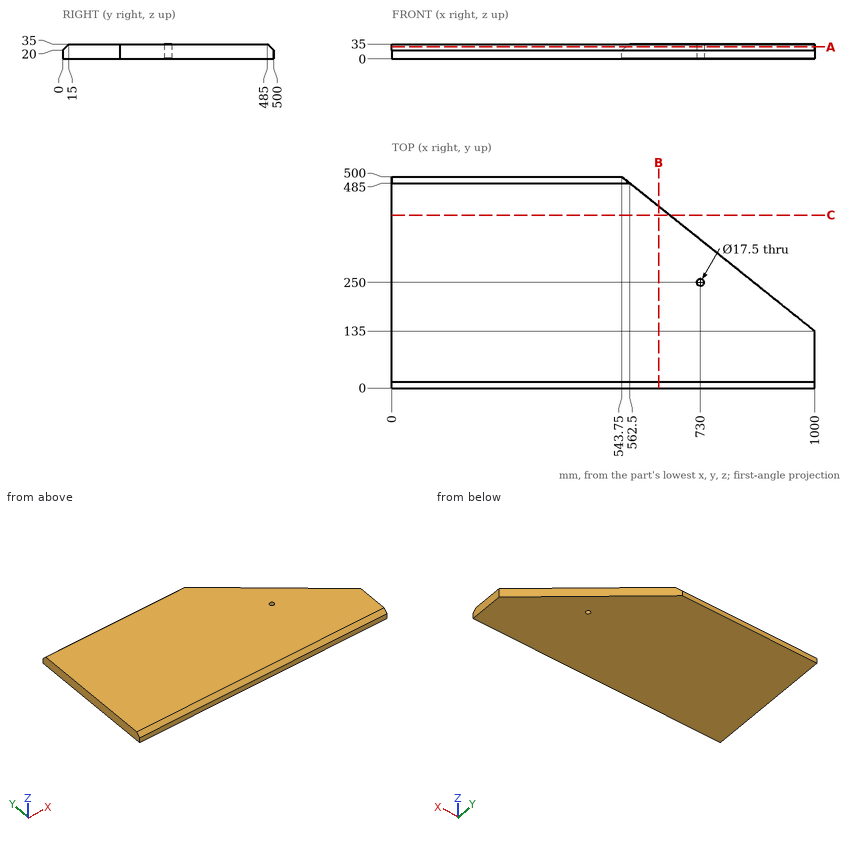
Could you check a few things on this drawing? It's one solid part, dimensions in mm from its lowest x, y, z. Coordinates: 2 decimals unless noted, no trailing zeros. Loops run counter-clockwise (first coordinate to the right, second up) from the corner with the lowest first, then second, coordinate; pieces in that order, holes last. Notation, with made-up numbers: (-40, 5.5) - (-24, 5.5) arc R22 ccw to (-24, 44.5) - close; hole circle Ø7 at (1.5, 16). An arc over 180 degrees is marked (long way). Return JSON: item names as keys, results as strings. Group by question number.
Item 1: If we section it at B-B on x = 631: Write out the boundary of the cut face in (y, z), and give its area (3 significant figures).
Item 2: I need wall thicknesses on line 1 (Y direction, x = 730, z = 18); line 2 (Y direction, x = 730, z = 21); line 3 (X direction, y = 231.5, z = 19.5) (3 decimals). Which ranges of each line are inside material? Lowest first, please. Write a range as from..to.
Item 3: Will these pins go through, and if not, where does the flat tip stop? P1, Ø14, axis at x = 730, y = 250, coming from the -Z side; P2, Ø6, axis at x = 426.5, z = 24.5, coming from the +Y side.
Item 4: If we section it at A-A on z = 28: Write out the boundary of the cut face in (x, y), and give its area (3 significant figures).
Item 5: If we section it at C-C on y = 409.5: Write out the boundary of the cut face in (x, z) (3 decimals).
Calculated:
{
 "1": {"outline": "(0, 0) - (430.2, 0) - (430.2, 35) - (15, 35) - (0, 20) - close", "area": "14,900 mm^2"},
 "2": {"line 1": "y = 0..241.25, 258.75..351", "line 2": "y = 1..241.25, 258.75..351", "line 3": "x = 0..879.375"},
 "3": {"P1": "passes through", "P2": "stops at y = 498.5"},
 "4": {"outline": "(0, 8) - (1000, 8) - (1000, 135) - (553.75, 492) - (0, 492) - close; hole circle Ø17.5 at (730, 250)", "area": "404,000 mm^2"},
 "5": {"outline": "(0, 0) - (656.875, 0) - (656.875, 35) - (0, 35) - close"}
}
